Here's how the part is built. I have some questions about the finished solid (model axes, mm). Face numbers are marked on the shaded views. A direction names the side the tool comes from. Round coordinates to 2 decimals unless told otherwise and drop trailing zeros. Order: outer loops, then holes, each group sorted by start corner. A loop starts at its lowest first (then second) coordinate and runs counter-clockwise, first axis right, second up. Notation, with made-up numbers: M 28.5,-10 L 76.5,-10 A20 cw 76.5,14 Z; hole C 29,-15.75 d8. An arc over 180 degrees is marked long. Answer as CSV lines item,"result". Start each with the question number.
```python
from build123d import *

# Parameters (mm, degrees)
EXTRUDE_368_DEPTH = 7.5
SKETCH_4_W        = 0.6
SKETCH_4_H        = 11.392304845
CHAMFER_1891_SIZE = 1.4
FILLET_1936_R     = 0.6


with BuildPart() as part:
    # 草图1 → Extrude 368 (new body)
    with BuildSketch(Plane(origin=(0, 0, 0), x_dir=(0, 0, -1), z_dir=(1, 0, 0))):
        Polygon((9, 5.196152423), (9, -5.196152423), (0, -10.392304845), (-9, -5.196152423), (-9, 5.196152423), (0, 10.392304845), align=None)
    extrude(amount=EXTRUDE_368_DEPTH)

    # 草图2 → 凸台-旋转1 (revolve)
    with BuildSketch(Plane.XY, mode=Mode.PRIVATE) as revolve_1_sk:
        Polygon((0, 0), (37.5, 0), (37.5, 4.4845), (37.5, 6), (0, 6), align=None)
    revolve(revolve_1_sk.sketch.rotate(Axis((0, 0, 0), (1, 0, 0)), 90), axis=Axis((0, 0, 0), (1, 0, 0)))

    # 草图3 → 切除-旋转1 (revolve, cut)
    with BuildSketch(Plane.XY):
        Polygon((0, 9), (3.690598923, 15.392304845), (3.690598923, 20.392304845), (-10, 20.392304845), (-10, 9), align=None)
    revolve(axis=Axis((0, 0, 0), (1, 0, 0)), mode=Mode.SUBTRACT)

    # 草图5 → 切除-旋转2 (revolve, cut)
    with BuildSketch(Plane.XY):
        Polygon((7.5, 9), (3.809401077, 15.392304845), (3.809401077, 20.392304845), (13.809401077, 20.392304845), (13.809401077, 9), align=None)
    revolve(axis=Axis((0, 0, 0), (1, 0, 0)), mode=Mode.SUBTRACT)

    # 草图4 → 切除-旋转3 (revolve, cut)
    with BuildSketch(Plane.XY, mode=Mode.PRIVATE) as cut_revolve_3_sk:
        with Locations((7.2, 14.696152423)):
            Rectangle(SKETCH_4_W, SKETCH_4_H)
    revolve(cut_revolve_3_sk.sketch.rotate(Axis((0, 0, 0), (1, 0, 0)), 270), axis=Axis((0, 0, 0), (1, 0, 0)), mode=Mode.SUBTRACT)

    # Chamfer 1891
    chamfer_1891_edges = [part.edges().sort_by_distance(p)[0] for p in [
        (37.5, 0, -6),
    ]]
    chamfer(chamfer_1891_edges, length=CHAMFER_1891_SIZE)

    # Fillet 1936
    fillet_1936_edges = [part.edges().sort_by_distance(p)[0] for p in [
        (7.5, 0, -6),
    ]]
    fillet(fillet_1936_edges, radius=FILLET_1936_R)


solid = part.part
```
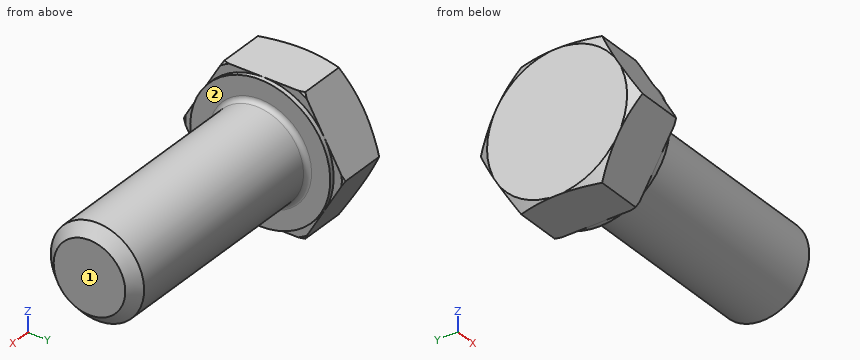
Item 1: If I drill on line 1 along X through (y, z) = (8.25, -3.5); line 2 along Z through (x, y) = (24, -3); line 3 along Y through (x, z) = (21.5, -0.25), over which ranges is the centre line in solid material (lowest first)?
Item 2: Which directions (+Z, -Z, +X, -X, +Y, -Y) give clear straight access to the entire face, cutting with the end or side of a thin tool? Please do the marked faces 1 and 2.
Item 3: For P1, Ø1, axis at y = -4, z = 0.5, coming from the -X side; P2, Ø1, axis at x = 27.5, y = 6, coming from the +Z side; P3, Ø2, axis at y = 5, z = 7.5, coming from the +X side; P4, Ø8, axis at x = 13, z = 1.5, coming from the -Y side, each with a flat end and sliding along its axis, tell me the tip position at first contact or that it passes through.
Item 4: If we section it at A-A on x = 6: Please give me the cut outline in (y, z).
Item 5: If we section it at B-B on x = 27.5: Please give me the cut outline in (y, z), and give its area (3 significant figures).
Geometry says:
1,line 1,"0 to 7.5"
1,line 2,"-5.2 to 5.2"
1,line 3,"-5.99 to 5.99"
2,face 1,"+Z, -Z, +X, +Y, -Y"
2,face 2,"+X"
3,P1,"x = 0"
3,P2,"z = 2.4"
3,P3,"x = 7.5"
3,P4,"y = -6"
4,outline,"M -10.39,0 L -5.2,-9 L 5.2,-9 L 10.39,0 L 5.2,9 L -5.2,9 Z"
5,outline,"C 0,0 d12"
5,area,"113 mm²"
